```python
from build123d import *

# Parameters (mm, degrees)
SKETCH_1_W      = 76
SKETCH_1_H      = 25
SKETCH_1_R      = 5
EXTRUDE_1_DEPTH = 7
SKETCH_2_W      = 12
SKETCH_2_H      = 25
EXTRUDE_2_DEPTH = 15


with BuildPart() as part:
    # 草图1 → 凸台-拉伸1 (new, symmetric)
    with BuildSketch(Plane.XY):
        Rectangle(SKETCH_1_W, SKETCH_1_H)
        with Locations((-26, 0)):
            Circle(SKETCH_1_R, mode=Mode.SUBTRACT)
    extrude(amount=EXTRUDE_1_DEPTH, both=True)

    # 草图2 → 凸台-拉伸2 (add)
    with BuildSketch(Plane.XY.offset(7)):
        with Locations((32, 0)):
            Rectangle(SKETCH_2_W, SKETCH_2_H)
    extrude(amount=EXTRUDE_2_DEPTH)


solid = part.part
```
Design review of the part built by this model. Coordinates are the model's own, in mm. A direction names the side the tool comes from. Give positions to 0.01 mm unless a question says otherwise; leave off trailing zeros. Write each loop counter-clockwise with the first axis right and the second up, starting at its lowest first coordinate (ties: lowest second). Pieces come first, ordered by that corner, then holes.
(1) Wall thickness on line 1 along Y through (x, z) = (-26, 4.25); line 2 along X through (y, z) = (8.5, 14); line 3 along Z through (x, y) = (-34, 8.5): over which ranges is each line inside the solid? List them lowest first.
Checked values:
line 1: y = -12.5 to -5, 5 to 12.5
line 2: x = 26 to 38
line 3: z = -7 to 7
(2) Add section C-C (z = -1.5). Give the boundary of the cut face in (x, y).
Checked values:
outline: (-38, -12.5) - (38, -12.5) - (38, 12.5) - (-38, 12.5) - close; hole circle Ø10 at (-26, 0)
(3) Mouldability with a two-part tool opening along Y and no side actions: class faces 1 (the face through (-6, 0, 7)), 2 (the face through (-1, -12.5, 1)), 3 (the face through (-31, 0, 0)) as +Y half, -Y half, draft (parallel to the pull), parting line (faces both ways), or undercut.
Checked values:
face 1: draft
face 2: -Y half
face 3: undercut
(4) Tool access review of faces 4 (the face through (-38, 0, 0)), 5 (the face through (26, 0, 14)): name each direction out of +Z, -Z, +X, -X, +Y, -Y from which nothing blocks a thin tool from reaching the whole face with its end or side.
Checked values:
face 4: +Z, -Z, -X, +Y, -Y
face 5: +Z, -X, +Y, -Y
(5) Add section B-B (y = 0). Give the boundary of the cut face in (x, z), and give its area (3 significant figures).
Checked values:
outline: (-38, -7) - (-31, -7) - (-31, 7) - (-38, 7) - close; (-21, -7) - (38, -7) - (38, 22) - (26, 22) - (26, 7) - (-21, 7) - close
area: 1,100 mm2
(6) Add section D-D (y = 9.75). Give the boundary of the cut face in (x, z), and give its area (3 significant figures).
Checked values:
outline: (-38, -7) - (38, -7) - (38, 22) - (26, 22) - (26, 7) - (-38, 7) - close
area: 1,240 mm2
(7) Clearance check with flat-ended pins moving along their axes: pin 1 Ø6 at (x, y) = (-26, 0) entering from -Z; pin 2 Ø12 at (x, y) = (-12, -3) entering from +Z. State where each tip first meets the part, or that it passes through.
Checked values:
pin 1: passes through
pin 2: stops at z = 7
(8) Add section A-A (x = -29). Give the boundary of the cut face in (y, z), and give its area (3 significant figures).
Checked values:
outline: (-12.5, -7) - (-4, -7) - (-4, 7) - (-12.5, 7) - close; (4, -7) - (12.5, -7) - (12.5, 7) - (4, 7) - close
area: 238 mm2
